```python
from build123d import *

# Parameters (mm, degrees)
BOSS_EXTRUDE1_DEPTH                                  = 5
HOLE_SIZE_BY_SOCKET_HEAD_CAP_SCREW_TYPE1_D           = 4.5
HOLE_SIZE_BY_SOCKET_HEAD_CAP_SCREW_TYPE1_DEPTH       = 16
HOLE_SIZE_BY_SOCKET_HEAD_CAP_SCREW_TYPE1_CBORE_D     = 8
HOLE_SIZE_BY_SOCKET_HEAD_CAP_SCREW_TYPE1_CBORE_DEPTH = 4.6
M4_TAPPED_HOLE1_D                                    = 3.3
M4_TAPPED_HOLE2_D                                    = 3.3
CHAMFER1_SIZE                                        = 0.5


with BuildPart() as part:
    # Sketch1 → Boss-Extrude1 (new, symmetric)
    with BuildSketch(Plane(origin=(0, 0, 0), x_dir=(0, 0, -1), z_dir=(1, 0, 0))):
        with BuildLine():
            Line((2, -9.440471387), (2, -18))
            Line((2, -18), (-2, -18))
            Line((-2, -18), (-2, -9.440471387))
            ThreePointArc((-2, -9.440471387), (-9.65, 0), (-2, 9.440471387))
            Line((-2, 9.440471387), (-2, 31.436443819))
            ThreePointArc((-2, 31.436443819), (-10.382706919, 29.739693963), (-18, 25.850531909))
            Line((-18, 25.850531909), (-18, 15))
            Line((-18, 15), (-27.699277969, 15))
            ThreePointArc((-27.699277969, 15), (0, -31.5), (27.699277969, 15))
            Line((27.699277969, 15), (18, 15))
            Line((18, 15), (18, 25.850531909))
            ThreePointArc((18, 25.850531909), (10.382706919, 29.739693963), (2, 31.436443819))
            Line((2, 31.436443819), (2, 9.440471387))
            ThreePointArc((2, 9.440471387), (9.65, 0), (2, -9.440471387))
        make_face()
    extrude(amount=BOSS_EXTRUDE1_DEPTH, both=True)

    # Hole size by socket head cap screw type1
    with Locations(Plane(origin=(0, 0, -18), x_dir=(-1, 0, 0), z_dir=(0, 0, -1))):
        with Locations((0, 21)):
            CounterBoreHole(HOLE_SIZE_BY_SOCKET_HEAD_CAP_SCREW_TYPE1_D / 2, HOLE_SIZE_BY_SOCKET_HEAD_CAP_SCREW_TYPE1_CBORE_D / 2, HOLE_SIZE_BY_SOCKET_HEAD_CAP_SCREW_TYPE1_CBORE_DEPTH, depth=HOLE_SIZE_BY_SOCKET_HEAD_CAP_SCREW_TYPE1_DEPTH)

    # M4 Tapped Hole1 (through all)
    with Locations(Plane(origin=(0, 0, 2), x_dir=(-1, 0, 0), z_dir=(0, 0, -1))):
        with Locations((0, 21)):
            Hole(M4_TAPPED_HOLE1_D / 2)

    # M4 Tapped Hole2 (through all)
    with Locations(Plane(origin=(5, 0, 0), x_dir=(0, 0, -1), z_dir=(1, 0, 0))):
        with Locations((20, 10), (20, -10), (-20, -10), (-20, 10)):
            Hole(M4_TAPPED_HOLE2_D / 2)

    # Chamfer1
    chamfer1_edges = [part.edges().sort_by_distance(p)[0] for p in [
        (5, 0, -9.65),
        (-5, 20.425265955, -18),
        (-5, 15, -22.849638984),
        (5, -13.720235693, -2),
        (-5, -31.5, 0),
        (-5, 15, 22.849638984),
        (-5, 20.425265955, 18),
        (-5, 29.739693963, 10.382706919),
        (-5, 20.438457603, 2),
        (-5, 0, 9.65),
        (-5, -13.720235693, 2),
        (5, -18, 0),
        (-5, -18, 0),
        (-5, -13.720235693, -2),
        (-5, 0, -9.65),
        (-5, 20.438457603, -2),
        (-5, 29.739693963, -10.382706919),
        (5, -13.720235693, 2),
        (5, 0, 9.65),
        (5, 20.438457603, 2),
        (5, 29.739693963, 10.382706919),
        (5, 20.425265955, 18),
        (5, 15, 22.849638984),
        (5, -31.5, 0),
        (5, 29.739693963, -10.382706919),
        (5, 15, -22.849638984),
        (5, 20.425265955, -18),
        (5, 10, 18.35),
        (-5, 10, 18.35),
        (5, -10, 18.35),
        (-5, -10, 18.35),
        (5, -10, -21.65),
        (-5, -10, -21.65),
        (5, 10, -21.65),
        (-5, 10, -21.65),
        (5, 20.438457603, -2),
    ]]
    chamfer(chamfer1_edges, length=CHAMFER1_SIZE)


solid = part.part
```
Input: part model. Units: mm. Frame: model coordinates. A direction names the side the tool comes from. Give positions to 0.01 mm unless a question says otherwise; leave off trailing zeros. Order: outer loops, then holes, each group sorted by start corner. A loop starts at its lowest first (then second) coordinate and runs counter-clockwise, first axis right, second up.
1. Cut plane A-A (z = 0). Return loops of the section in (x, y), and give its area (4 significant figures).
Computed:
outline: (-5, -31) - (-4.5, -31.5) - (4.5, -31.5) - (5, -31) - (5, -18.5) - (4.5, -18) - (-4.5, -18) - (-5, -18.5) - close
area: 134.5 mm2
2. Set-up query: faces 1 (the face through (0, 15, 23)), 2 (the face through (0, 18, -2)), 3 (the face through (5, 7.3, 7.3)), 4 (the face through (0, 15, -23)), 5 (the face through (-4.635, -0.187, 9.784)). Return all of +Z, -Z, +X, -X, +Y, -Y with unobstructed straight access to the full face (end or side cutting, diameter ignored); none if empty.
Computed:
face 1: +Z, +X, -X, +Y
face 2: +X, -X, +Y
face 3: +Z, -Z, +X, +Y, -Y
face 4: -Z, +X, -X, +Y
face 5: -X
3. Line query: probe 1 along Y at (x, z) = (0, 8.5); probe 2 along Z at (x, y) = (2, 22.5); probe 3 along Y at (x, z) = (0, -21.5). Output: solid intervals per line, ascending.
Computed:
probe 1: y = -30.33 to -4.57, 4.57 to 19.35, 22.65 to 30.33
probe 2: z = -13.4 to -2, 2 to 18
probe 3: y = -23.02 to -10.69, -9.31 to 9.31, 10.69 to 15
4. Draft query along Y for faces 6 (the face through (4.858, -31.129, 0.901)), 7 (the face through (-5, 7.3, 7.3)), 8 (the face through (-0.488, 18.804, -7.62)). Return one class per face: released by +Y, released by -Y, zero draft, split by the parting line, or undercut.
Computed:
face 6: split by the parting line
face 7: zero draft
face 8: undercut
5. Pin query (flat end, axial travel): pin 1 Ø5 at (x, y) = (-3, -21.5) entering from -Z; pin 2 Ø1 at (x, z) = (3.5, 9) entering from -Y; pin 3 Ø6 at (x, y) = (-1, -7) entering from -Z (3 decimals). Return the tip coordinate at first contact, or that it passes through.
Computed:
pin 1: stops at z = -25.12
pin 2: stops at y = -30.33
pin 3: stops at z = -31.245
6. Cut plane C-C (z = 8). State how many separate pieces and enclosed holes the cut face has, and give its area (3 significant figures).
Computed:
separate pieces: 2
enclosed holes: 1
area: 491 mm2
7. Cut plane B-B (x = 3). Return loops of the section in (y, z).
Computed:
outline: (-18, -2) - (-18, 2) - (-9.44, 2) arc R9.65 cw to (9.44, 2) - (31.44, 2) arc R31.5 ccw to (25.85, 18) - (15, 18) - (15, 27.7) arc R31.5 ccw (long way) to (15, -27.7) - (15, -18) - (18.35, -18) - (18.35, -13.4) - (23.65, -13.4) - (23.65, -18) - (25.85, -18) arc R31.5 ccw to (31.44, -2) - (9.44, -2) arc R9.65 cw to (-9.44, -2) - close; hole circle Ø3.3 at (-10, -20); hole circle Ø3.3 at (-10, 20); hole circle Ø3.3 at (10, -20); hole circle Ø3.3 at (10, 20)
